For this review, take the finished solid that the model builds, in its own axes (mm). Face numbers are marked on the shaded views. Round coordinates to 2 decimals unless told otherwise and drop trailing zeros. Loops run counter-clockwise (first coordinate to the right, second up) from the corner with the lowest first, then second, coordinate; pieces in that order, holes last.
1) Take a section at A-A (x = -1). State the section outline as (y, z) points, then the cut area to 3 significant figures.
2) Wall thickness on L1, parallel to X at y = 2, z = 3; L2, parallel to Y at x = 0.5, z = 2.5; L3, parallel to X at y = -0.5, z = 2.5: over which ranges is each line inside the solid? List them lowest first.
3) Take a section at B-B (z = 4). State the section outline as (x, y) points, then the cut area to 3 significant figures.
4) Take a section at C-C (y = 3). State the section outline as (x, z) points, then the cut area to 3 significant figures.
5) Mouldability with a two-part tool opening along X and no side actions: class the marked faces 1, 2 and 3 as pulls with the +X half, pulls with the -X half, needs draft (parallel to the pull), parting line crosses it, or undercut.
6) Take a section at D-D (y = -4.25). State the section outline as (x, z) points.
7) Insertion check: pin 1 (4 mm diameter, centred on x = 7.32, y = 3.57, fed in from -Z); pin 2 (1 mm diameter, centred on y = -16.5, z = 1.5, fed in from +X); pin 3 (1.5 mm diameter, centred on x = -13, y = -14, fed in from -Z); pin 4 (1 mm diameter, centred on y = 2, z = 4.5, fed in from -X). Each pin has a flat end and moves straight along its axis. Give the tip position at first contact, or say it passes through.
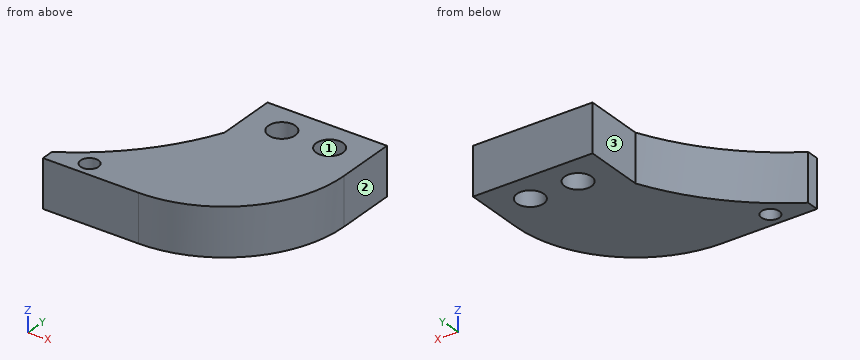
```python
from build123d import *

# Parameters (mm, degrees)
EXTRUDE_1_DEPTH     = 8
SKETCH_2_R          = 1.5
SKETCH_2_R_2        = 2.25
CUT_EXTRUDE_1_DEPTH = 33.213594803


with BuildPart() as part:
    # 草图1 → 凸台-拉伸1 (new body)
    with BuildSketch(Plane.XY):
        with BuildLine():
            Line((-6.680497925, 8.56846473), (13.319502075, 8.56846473))
            Line((13.319502075, 8.56846473), (13.319502075, -1.43153527))
            ThreePointArc((13.319502075, -1.43153527), (7.461637698, -15.573670893), (-6.680497925, -21.43153527))
            Line((-6.680497925, -21.43153527), (-22.680497925, -21.43153527))
            Line((-22.680497925, -21.43153527), (-22.680497925, -19.349484524))
            ThreePointArc((-22.680497925, -19.349484524), (-13.301383699, -11.622002815), (-6.680497925, -1.43153527))
            Line((-6.680497925, -1.43153527), (-6.680497925, 8.56846473))
        make_face()
    extrude(amount=EXTRUDE_1_DEPTH)

    # 草图2 → 切除-拉伸1 (cut, through all)
    with BuildSketch(Plane(origin=(0, 0, 0), x_dir=(-1, 0, 0), z_dir=(0, 0, -1))):
        with Locations((16.680497925, -18.93153527)):
            Circle(SKETCH_2_R)
        with Locations((0.680497925, 3.56846473)):
            Circle(SKETCH_2_R_2)
        with Locations((-7.319502075, 3.56846473)):
            Circle(SKETCH_2_R_2)
    extrude(amount=-CUT_EXTRUDE_1_DEPTH, mode=Mode.SUBTRACT)


solid = part.part
```
Response:
1. outline: (-20.61, 0) - (1.34, 0) - (1.34, 8) - (-20.61, 8) - close; (5.8, 0) - (8.57, 0) - (8.57, 8) - (5.8, 8) - close
1. area: 198 mm2
2. L1: x = -6.68 to -2.29, 0.93 to 5.71, 8.93 to 13.32
2. L2: y = -20.1 to 1.65, 5.48 to 8.57
2. L3: x = -6.68 to 13.32
3. outline: (-22.68, -21.43) - (-6.68, -21.43) arc R20 ccw to (13.32, -1.43) - (13.32, 8.57) - (-6.68, 8.57) - (-6.68, -1.43) arc R39.94 cw to (-22.68, -19.35) - close; hole circle Ø3 at (-16.68, -18.93); hole circle Ø4.5 at (-0.68, 3.57); hole circle Ø4.5 at (7.32, 3.57)
3. area: 622 mm2
4. outline: (-6.68, 0) - (-2.86, 0) - (-2.86, 8) - (-6.68, 8) - close; (1.5, 0) - (5.14, 0) - (5.14, 8) - (1.5, 8) - close; (9.5, 0) - (13.32, 0) - (13.32, 8) - (9.5, 8) - close
4. area: 90.3 mm2
5. face 1: undercut
5. face 2: pulls with the +X half
5. face 3: pulls with the -X half
6. outline: (-8.09, 0) - (13.12, 0) - (13.12, 8) - (-8.09, 8) - close
7. pin 1: passes through
7. pin 2: stops at x = 7.02
7. pin 3: stops at z = 0
7. pin 4: stops at x = -6.68
